Input: part model. Units: mm. Frame: model coordinates. Face numbers are marked on the shaded views. A direction names the side the tool comes from. Give positions to 0.01 mm unless a question says otherwise; leave off trailing zeros. Order: outer loops, then holes, each group sorted by start corner. A loop starts at its lowest first (then second) coordinate and runs counter-clockwise, first axis right, second up. Notation, with made-up numbers: (-36, 30) - (13, 30) arc R34 ccw to (13, 68) - close; hole circle Ø7 at (66, -26.75). An arc over 180 degrees is marked (long way). Use a Markdown table: item, result.
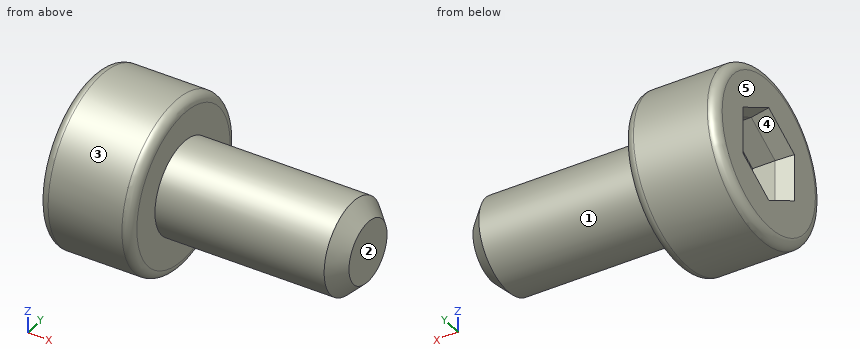
from build123d import *

# Parameters (mm, degrees)
CUT_EXTRUDE1_DEPTH = 1.3
FILLET1_R          = 0.3
CHAMFER1_SIZE      = 0.1
CHAMFER1_SIZE2     = 0.567128182
CHAMFER2_SIZE      = 0.5


with BuildPart() as part:
    # Sketch1 → Revolve1 (revolve)
    with BuildSketch(Plane.XY, mode=Mode.PRIVATE) as revolve1_sk:
        Polygon((0, 0), (0, 2.75), (3, 2.75), (3, 1.5), (9, 1.5), (9, 0), align=None)
    revolve(revolve1_sk.sketch.rotate(Axis((-4.709244637, 0, 0), (1, 0, 0)), 180), axis=Axis((-4.709244637, 0, 0), (1, 0, 0)))

    # Sketch4 → Cut-Extrude1 (cut)
    with BuildSketch(Plane.ZY):
        Polygon((-1.443375673, 0), (-0.721687836, -1.25), (0.721687836, -1.25), (1.443375673, 0), (0.721687836, 1.25), (-0.721687836, 1.25), align=None)
    extrude(amount=-CUT_EXTRUDE1_DEPTH, mode=Mode.SUBTRACT)

    # Fillet1
    fillet1_edges = [part.edges().sort_by_distance(p)[0] for p in [
        (3, 2.75, 0),
        (0, 2.75, 0),
    ]]
    fillet(fillet1_edges, radius=FILLET1_R)

    # Chamfer1
    chamfer1_edges = [part.edges().sort_by_distance(p)[0] for p in [
        (0, 0.625, -1.082531755),
        (0, -0.625, -1.082531755),
        (0, -1.25, 0),
        (0, -0.625, 1.082531755),
        (0, 0.625, 1.082531755),
        (0, 1.25, 0),
    ]]
    chamfer1_side = [part.faces().sort_by_distance(p)[0] for p in [
        (0, 2.380703535, 0),
    ]]
    chamfer(chamfer1_edges, length=CHAMFER1_SIZE, length2=CHAMFER1_SIZE2, reference=chamfer1_side[0])

    # Chamfer2
    chamfer2_edges = [part.edges().sort_by_distance(p)[0] for p in [
        (9, 1.5, 0),
    ]]
    chamfer(chamfer2_edges, length=CHAMFER2_SIZE)


solid = part.part
1. Section query A-A (z = 0). Return loops of the section in (x, y), then the cut area to 3 significant figures.
Response:
| item | result |
|---|---|
| outline | (0, -2.45) arc R0.3 ccw to (0.3, -2.75) - (2.7, -2.75) arc R0.3 ccw to (3, -2.45) - (3, -1.5) - (8.5, -1.5) - (9, -1) - (9, 1) - (8.5, 1.5) - (3, 1.5) - (3, 2.45) arc R0.3 ccw to (2.7, 2.75) - (0.3, 2.75) arc R0.3 ccw to (0, 2.45) - (0, 1.35) - (0.57, 1.25) - (1.3, 1.25) - (1.3, -1.25) - (0.57, -1.25) - (0, -1.35) - close |
| area | 30.9 mm^2 |
2. Section query B-B (x = 2.5). Return loops of the section in (y, z), then the cut area to 3 significant figures.
Response:
| item | result |
|---|---|
| outline | circle Ø5.5 at (0, 0) |
| area | 23.8 mm^2 |
3. Pin query (flat end, axial travel): pin 1 (1 mm diameter, centred on x = 1, z = 2, fed in from -Y). Return the tip coordinate at first contact, or that it passes through.
Response:
| item | result |
|---|---|
| pin 1 | stops at y = -2.3 |
4. Mould query, pull axis Z, two halves, no side actions, for the marked faces 3, 4 and 5. Classes: pulls with the +Z half, pulls with the -Z half, needs draft (parallel to the pull), parting line crosses it, or undercut.
Response:
| item | result |
|---|---|
| face 3 | parting line crosses it |
| face 4 | undercut |
| face 5 | needs draft |
5. Set-up query: the marked faces 1 and 2. Return all of +Z, -Z, +X, -X, +Y, -Y with unobstructed straight access to the full face (end or side cutting, diameter ignored); none if empty.
Response:
| item | result |
|---|---|
| face 1 | +X |
| face 2 | +Z, -Z, +X, +Y, -Y |
6. Section query C-C (x = 5.75). Return loops of the section in (y, z).
Response:
| item | result |
|---|---|
| outline | circle Ø3 at (0, 0) |
7. Material intervals for line 1 along X through (y, z) = (0.8, 0.35); line 2 along Z through (x, y) = (1, -0.6); line 3 along Y through (x, z) = (1.25, 0.2), sorted ascending.
Response:
| item | result |
|---|---|
| line 1 | x = 1.3 to 9 |
| line 2 | z = -2.68 to -1.1, 1.1 to 2.68 |
| line 3 | y = -2.74 to -1.25, 1.25 to 2.74 |
